Can you work these out from the drawing? Everything is in mm from the part's minimum corner. Coordinates: 2 decimals unless noted, no trailing zeros. Order: outer loops, then holes, each group sorted by start corner. A loop starts at its lowest first (then second) coordinate and runs counter-clockwise, first axis right, second up. Notation, with made-up numbers: (76, 35) - (86, 35) arc R26 cw to (86, 57) - close; hole circle Ø6 at (52, 70). An arc over 180 degrees is marked (long way). One line per item, written item: value.
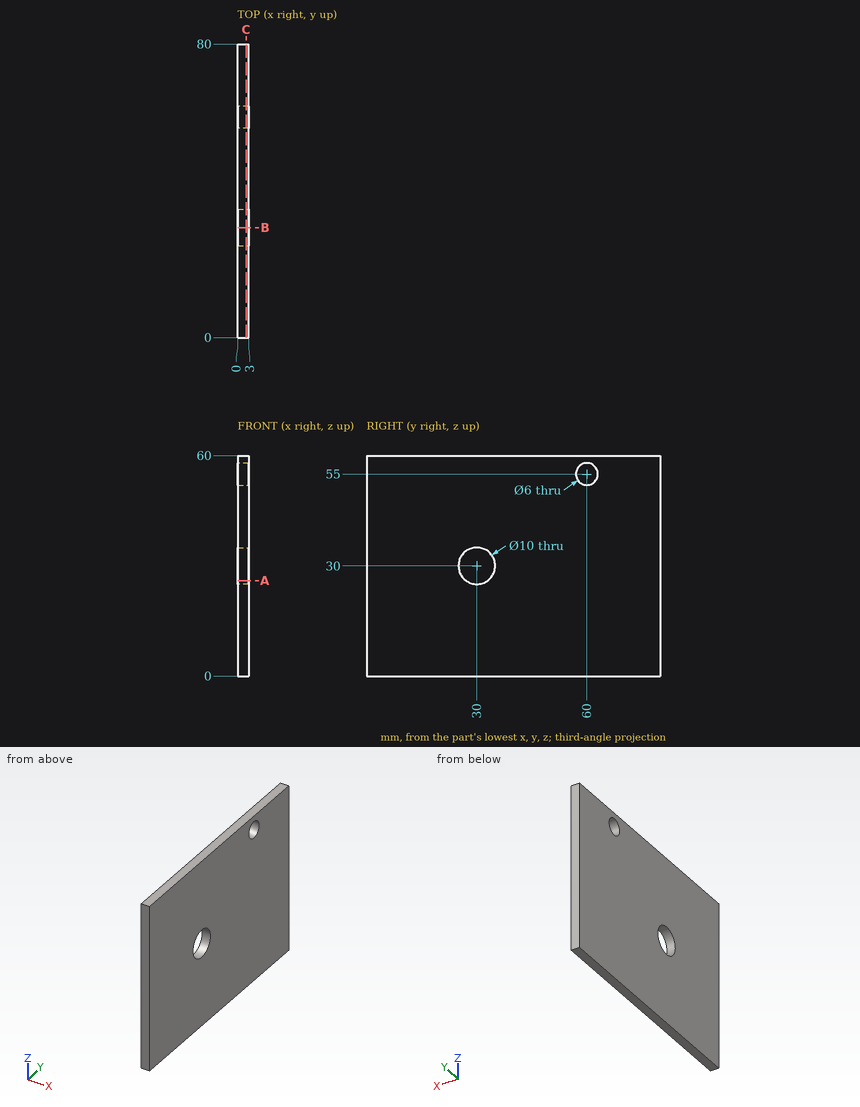
Item 1: I want a section at B-B on y = 30. Please give me the cut outline in (x, z), then the cut area to 3 significant figures.
Conclusion:
outline: (0, 0) - (3, 0) - (3, 25) - (0, 25) - close; (0, 35) - (3, 35) - (3, 60) - (0, 60) - close
area: 150 mm²
Item 2: I want a section at C-C on x = 2.3. Please give me the cut outline in (y, z), then the cut area to 3 significant figures.
Conclusion:
outline: (0, 0) - (80, 0) - (80, 60) - (0, 60) - close; hole circle Ø10 at (30, 30); hole circle Ø6 at (60, 55)
area: 4,690 mm²
Item 3: If I drill on probe 1 along Y at (x, z) = (1.6, 30); probe 2 along Z at (x, y) = (1.55, 34); probe 3 along Y at (x, z) = (1.05, 55.5), over which ranges is the centre line in solid material (lowest first)?
Conclusion:
probe 1: 0 to 25, 35 to 80
probe 2: 0 to 27, 33 to 60
probe 3: 0 to 57.04, 62.96 to 80
Item 4: I want a section at A-A on z = 26. Please give me the cut outline in (x, y).
Conclusion:
outline: (0, 0) - (3, 0) - (3, 27) - (0, 27) - close; (0, 33) - (3, 33) - (3, 80) - (0, 80) - close
